Geometry check sheet. Reference: the model listing, model coordinates, mm. A direction names the side the tool comes from. Give positions to 0.01 mm unless a question says otherwise; leave off trailing zeros. Loops run counter-clockwise (first coordinate to the right, second up) from the corner with the lowest first, then second, coordinate; pieces in that order, holes last.
1. Release check for a two-part mould opening along Y. For faces 1 (the flat face through (-29.2, 9, -18)), 2 (the flat face through (0, 0, -1)), 3 (the cylindrical face through (13.071, 0.811, 41.312)), 4 (the flat face through (-21, 15.3, 18)) record: +Y half, -Y half, draft (parallel to the pull), parting line (faces both ways), or undercut.
2. Go/stop test with flat-tipped pins: pin 1 Ø5 at (x, z) = (0, 39.5) entering from +Y; pin 2 Ø4 at (x, y) = (-19.5, 8.5) entering from +Z; pin 3 Ø6 at (y, z) = (6.5, -22.5) entering from +X; pin 4 Ø12 at (x, z) = (-19, -22) entering from -Y. Record where each tip stops, or that it passes through.
3. Cross-section at B-B, the plane y = 6.75. Record the cut outline in (x, z).
4. Tool access check on faces 5 (the flat face through (-21, 8, 10.1)), 6 (the flat face through (-21, 8, -25.9)), 7 (the flat face through (-11.7, 9, 18)). Record the directions out of +Z, -Z, +X, -X, +Y, -Y that give a thin tool (end or side, any length) a straight path to the whole face; none if there is none.
5. Cross-section at C-C, the plane x = 12.5. Record the cut outline in (y, z).
6. Cross-section at D-D, the plane x = -21. Record the cut outline in (y, z), plus the area to 3 significant figures.
7. Cross-section at A-A, the plane z = 39.5. Record the cut outline in (x, y), plus the area to 3 significant figures.
8. Material ranges on L1, parallel to X at y = 0.75, z = -39.5; L2, parallel to Z at x = -15.5, y = 6.75; L3, parallel to Y at x = -8.5, z = -7, recorded low to high.
from build123d import *

# Parameters (mm, degrees)
SKETCH_1_W          = 60.4
SKETCH_1_H          = 89.7
EXTRUDE_1_DEPTH     = 1.6
SKETCH_2_R          = 1.9
CUT_EXTRUDE_1_DEPTH = 1.6
SKETCH_3_W          = 15.8
SKETCH_3_H          = 13.7
EXTRUDE_2_DEPTH     = 18.5
SKETCH_4_W          = 51.8
SKETCH_4_H          = 0.2
CUT_EXTRUDE_2_DEPTH = 1
SKETCH_5_W          = 12.792520148
SKETCH_5_H          = 10.634773198
SKETCH_5_W_2        = 12.994853118
SKETCH_5_H_2        = 11.260006872
CUT_EXTRUDE_3_DEPTH = 1


with BuildPart() as part:
    # 草图1 → 凸台-拉伸1 (new body)
    with BuildSketch(Plane(origin=(0, 0, 0), x_dir=(1, 0, 0), z_dir=(0, 1, 0))):
        Rectangle(SKETCH_1_W, SKETCH_1_H)
    extrude(amount=EXTRUDE_1_DEPTH)

    # 草图2 → 切除-拉伸1 (cut)
    with BuildSketch(Plane(origin=(0, 1.6, 0), x_dir=(1, 0, 0), z_dir=(0, 1, 0))):
        with Locations(Location((-12.5, -39.5, 0), (0, 0, 270))):
            Circle(SKETCH_2_R)
        with Locations(Location((12.5, -39.5, 0), (0, 0, 270))):
            Circle(SKETCH_2_R)
        with Locations(Location((-12.5, 39.5, 0), (0, 0, 270))):
            Circle(SKETCH_2_R)
        with Locations(Location((12.5, 39.5, 0), (0, 0, 270))):
            Circle(SKETCH_2_R)
        with Locations(Location((0, 39.5, 0), (0, 0, 270))):
            Circle(SKETCH_2_R)
        with Locations(Location((0, -39.5, 0), (0, 0, 270))):
            Circle(SKETCH_2_R)
    extrude(amount=-CUT_EXTRUDE_1_DEPTH, mode=Mode.SUBTRACT)

    # 草图3 → 凸台-拉伸2 (add)
    with BuildSketch(Plane.ZY.offset(30.2)):
        with Locations((18, 8.45)):
            Rectangle(SKETCH_3_W, SKETCH_3_H)
        with Locations((-18, 8.45)):
            Rectangle(SKETCH_3_W, SKETCH_3_H)
    extrude(amount=-EXTRUDE_2_DEPTH)

    # 草图4 → 切除-拉伸2 (cut)
    with BuildSketch(Plane.ZY.offset(30.2)):
        with Locations((0, 1.7)):
            Rectangle(SKETCH_4_W, SKETCH_4_H)
    extrude(amount=-CUT_EXTRUDE_2_DEPTH, mode=Mode.SUBTRACT)

    # 草图5 → 切除-拉伸3 (cut)
    with BuildSketch(Plane.ZY.offset(30.2)):
        with Locations((18, 8.55)):
            Rectangle(SKETCH_5_W, SKETCH_5_H)
        with Locations((-18, 8.55)):
            Rectangle(SKETCH_5_W_2, SKETCH_5_H_2)
    extrude(amount=-CUT_EXTRUDE_3_DEPTH, mode=Mode.SUBTRACT)


solid = part.part
Result:
1. face 1: undercut
1. face 2: -Y half
1. face 3: draft
1. face 4: +Y half
2. pin 1: stops at y = 1.6
2. pin 2: stops at z = 25.9
2. pin 3: stops at x = -11.7
2. pin 4: stops at y = 0
3. outline: (-30.2, -25.9) - (-11.7, -25.9) - (-11.7, -10.1) - (-30.2, -10.1) - (-30.2, -11.5) - (-29.2, -11.5) - (-29.2, -24.5) - (-30.2, -24.5) - close; (-30.2, 10.1) - (-11.7, 10.1) - (-11.7, 25.9) - (-30.2, 25.9) - (-30.2, 24.4) - (-29.2, 24.4) - (-29.2, 11.6) - (-30.2, 11.6) - close
4. face 5: +X, -X, +Y
4. face 6: -Z, +X, -X, +Y
4. face 7: +Z, -Z, +X, +Y
5. outline: (0, -44.85) - (1.6, -44.85) - (1.6, -41.4) - (0, -41.4) - close; (0, -37.6) - (1.6, -37.6) - (1.6, 37.6) - (0, 37.6) - close; (0, 41.4) - (1.6, 41.4) - (1.6, 44.85) - (0, 44.85) - close
6. outline: (0, -44.85) - (1.6, -44.85) - (1.6, -25.9) - (15.3, -25.9) - (15.3, -10.1) - (1.6, -10.1) - (1.6, 10.1) - (15.3, 10.1) - (15.3, 25.9) - (1.6, 25.9) - (1.6, 44.85) - (0, 44.85) - close
6. area: 576 mm2
7. outline: (-30.2, 0) - (-14.4, 0) - (-14.4, 1.6) - (-30.2, 1.6) - close; (-10.6, 0) - (-1.9, 0) - (-1.9, 1.6) - (-10.6, 1.6) - close; (1.9, 0) - (10.6, 0) - (10.6, 1.6) - (1.9, 1.6) - close; (14.4, 0) - (30.2, 0) - (30.2, 1.6) - (14.4, 1.6) - close
7. area: 78.4 mm2
8. L1: x = -30.2 to -14.4, -10.6 to -1.9, 1.9 to 10.6, 14.4 to 30.2
8. L2: z = -25.9 to -10.1, 10.1 to 25.9
8. L3: y = 0 to 1.6
